For this review, take the finished solid that the model builds, in its own axes (mm). Coordinates: 2 decimals unless noted, no trailing zeros. Write each loop counter-clockwise with the first axis right and the second up, starting at its lowest first coordinate (ties: lowest second). Pieces come first, ordered by that corner, then holes. Notation, with made-up numbers: (62.5, 36) -> (102.5, 36) arc R21 cw to (102.5, 66) -> close; hole circle Ø6 at (-12.5, -17). An arc over 180 degrees is marked (long way). One line per item, written item: value. Start each with the question number.
1) For probe 1 along Y at (x, z) = (0, 3.5); probe 2 along Y at (x, z) = (-13, 10.5); probe 3 along Y at (x, z) = (1.5, 7), list the stretches that pass through material, from the lowest coordinate up. Write a range as from..to.
2) Mouldability with a two-part tool opening along Y and no side actions: class faces 1 (the flat face through (-20, 5, 7)), 2 (the cylindrical face through (3.92, -207.54, 6.9)), 3 (the cylindrical face through (0, -220, 7)) as released by +Y, released by -Y, zero draft, split by the parting line, or undercut.
3) Add section B-B (x = 0). State the section outline as (y, z) points, and give its area (3 significant figures).
4) Add section A-A (z = 8.25). State the section outline as (x, y) points, and give its area (3 significant figures).
5) For pin 1 Ø17 at (x, y) = (0, 120) entering from -Z, flat-tipped, find the tip position at first contact; note if it passes through.
from build123d import *

# Parameters (mm, degrees)
SKETCH_1_R          = 9.5
SKETCH_1_R_2        = 8.5
EXTRUDE_1_DEPTH     = 14
SKETCH_2_R          = 5
CUT_EXTRUDE_1_DEPTH = 20


with BuildPart() as part:
    # 草图1 → 凸台-拉伸1 (new body)
    with BuildSketch(Plane.XY):
        with BuildLine():
            Line((-15, 220), (15, 220))
            ThreePointArc((15, 220), (18.535533906, 218.535533906), (20, 215))
            Line((20, 215), (20, -200))
            ThreePointArc((20, -200), (0, -220), (-20, -200))
            Line((-20, -200), (-20, 215))
            ThreePointArc((-20, 215), (-18.535533906, 218.535533906), (-15, 220))
        make_face()
        with Locations((0, 120)):
            Circle(SKETCH_1_R, mode=Mode.SUBTRACT)
        with Locations((0, -200)):
            Circle(SKETCH_1_R_2, mode=Mode.SUBTRACT)
    extrude(amount=EXTRUDE_1_DEPTH)

    # 草图2 → 切除-拉伸1 (cut)
    with BuildSketch(Plane(origin=(0, 0, 0), x_dir=(-1, 0, 0), z_dir=(0, 0, -1))):
        with Locations((12, 212)):
            Circle(SKETCH_2_R)
    extrude(amount=-CUT_EXTRUDE_1_DEPTH, mode=Mode.SUBTRACT)


solid = part.part
Numbers:
1. probe 1: -220..-208.5, -191.5..110.5, 129.5..220
1. probe 2: -215.2..207.1, 216.9..220
1. probe 3: -219.94..-208.37, -191.63..110.62, 129.38..220
2. face 1: zero draft
2. face 2: undercut
2. face 3: released by -Y
3. outline: (-220, 0) -> (-208.5, 0) -> (-208.5, 14) -> (-220, 14) -> close; (-191.5, 0) -> (110.5, 0) -> (110.5, 14) -> (-191.5, 14) -> close; (129.5, 0) -> (220, 0) -> (220, 14) -> (129.5, 14) -> close
3. area: 5,660 mm²
4. outline: (-20, -200) arc R20 ccw to (20, -200) -> (20, 215) arc R5 ccw to (15, 220) -> (-15, 220) arc R5 ccw to (-20, 215) -> close; hole circle Ø10 at (-12, 212); hole circle Ø19 at (0, 120); hole circle Ø17 at (0, -200)
4. area: 16,800 mm²
5. pin 1: through
